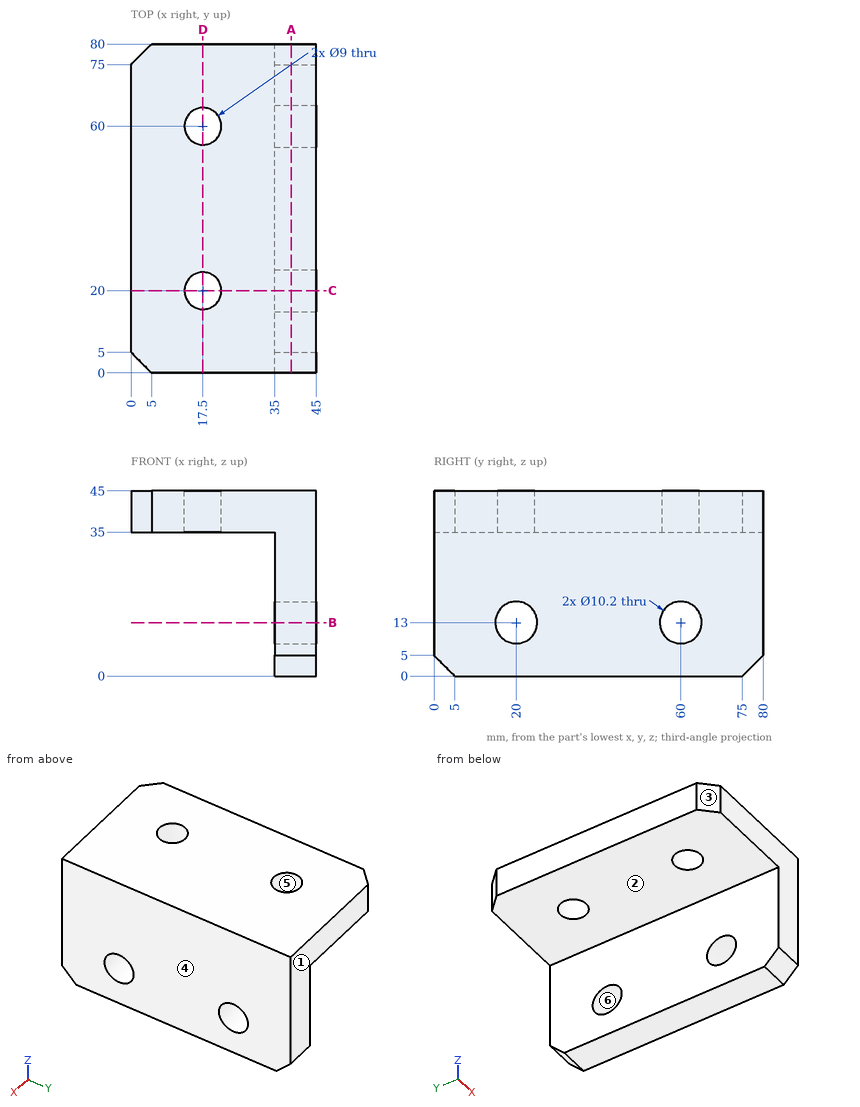
Can you work these out from the drawing? Everything is in mm from the part's minimum corner. A direction names the side the tool comes from. Give positions to 0.01 mm unless a question says otherwise; leave off trailing zeros. Loops run counter-clockwise (first coordinate to the right, second up) from the corner with the lowest first, then second, coordinate; pieces in that order, holes last. Notation, with made-up numbers: (-4, 33.25) -> (6, 33.25) arc R28 ccw to (6, 67.25) -> close; hole circle Ø8 at (-16.5, -31.75). An arc over 180 degrees is marked (long way). Return JSON: item names as keys, results as strings.
Q1. I want a section at B-B, the plane z = 13. List the corners of the cut face in (x, y) for me.
Checks:
{"outline": "(35, 0) -> (45, 0) -> (45, 14.9) -> (35, 14.9) -> close; (35, 25.1) -> (45, 25.1) -> (45, 54.9) -> (35, 54.9) -> close; (35, 65.1) -> (45, 65.1) -> (45, 80) -> (35, 80) -> close"}
Q2. We'd pull the mould along Y, two halves only. Please class the marked faces 3, 4, 5 and 6: released by +Y, released by -Y, zero draft, split by the parting line, or undercut.
Checks:
{"face 3": "released by -Y", "face 4": "zero draft", "face 5": "undercut", "face 6": "undercut"}
Q3. I want a section at A-A, the plane x = 39. List the corners of the cut face in (y, z) for me.
Checks:
{"outline": "(0, 5) -> (5, 0) -> (75, 0) -> (80, 5) -> (80, 45) -> (0, 45) -> close; hole circle Ø10.2 at (20, 13); hole circle Ø10.2 at (60, 13)"}
Q4. I want a section at D-D, the plane x = 17.5. List the corners of the cut face in (y, z) for me.
Checks:
{"outline": "(0, 35) -> (15.5, 35) -> (15.5, 45) -> (0, 45) -> close; (24.5, 35) -> (55.5, 35) -> (55.5, 45) -> (24.5, 45) -> close; (64.5, 35) -> (80, 35) -> (80, 45) -> (64.5, 45) -> close"}
Q5. For pin 1 Ø8 at (x, y) = (11.5, 41.5) entering from -Z; pin 2 Ø12 at (y, z) = (70.5, 19.5) entering from -X, each with a flat end and sliding along its axis, tell me the tip position at first contact or that it passes through.
Checks:
{"pin 1": "stops at z = 35", "pin 2": "stops at x = 35"}
Q6. On a 3-axis mill with a long thin cutter (end or side, diameter ignored), from which of +Z, -Z, +X, -X, +Y, -Y can I reach the whole of each face in a straight line? I mean the marked faces 1 and 2. Say none if no direction works.
Checks:
{"face 1": "+Z, -Z, +X, -X, +Y", "face 2": "-Z, -X, +Y, -Y"}
Q7. I want a section at C-C, the plane y = 20. List the corners of the cut face in (x, z) for me, then the cut area to 3 significant figures.
Checks:
{"outline": "(0, 35) -> (13, 35) -> (13, 45) -> (0, 45) -> close; (22, 35) -> (35, 35) -> (35, 18.1) -> (45, 18.1) -> (45, 45) -> (22, 45) -> close; (35, 0) -> (45, 0) -> (45, 7.9) -> (35, 7.9) -> close", "area": "608 mm2"}
Q8. I need wall thicknesses on probe 1 along Y at (x, z) = (40, 13); probe 2 along Y at (x, z) = (17.5, 41.75); probe 3 along Z at (x, y) = (29, 27). Which ranges of each line are inside material? Lowest first, please.
Checks:
{"probe 1": "y = 0 to 14.9, 25.1 to 54.9, 65.1 to 80", "probe 2": "y = 0 to 15.5, 24.5 to 55.5, 64.5 to 80", "probe 3": "z = 35 to 45"}
